Here's how the part is built. I have some questions about the finished solid (model axes, mm). Face numbers are marked on the shaded views. A direction names the side the tool comes from. Round coordinates to 2 decimals unless told otherwise and drop trailing zeros. Loops run counter-clockwise (first coordinate to the right, second up) from the corner with the lowest first, then second, coordinate; pieces in that order, holes last. Notation, with made-up numbers: (87.5, 84.25) - (116.5, 84.25) arc R13 cw to (116.5, 95.25) - close; hole circle Ø4 at (-17.75, -16.75). An arc over 180 degrees is marked (long way). Answer as a JSON object with one key per item and string values. Group by question number.
1) If we mould it in two halves opening along X, with no side actions, what happens to the marked faces 1, 2, 3 and 4? For each: pulls with the +X half, pulls with the -X half, needs draft (parallel to the pull), parting line crosses it, or undercut.
2) I want a section at C-C, the plane z = 27. Please give me the cut outline in (x, y), then the cut area to 3 significant figures.
3) I want a section at B-B, the plane z = 100. Please give me the cut outline in (x, y), then the cut area to 3 significant figures.
4) I want a section at A-A, the plane x = 18.5. Please give me the cut outline in (y, z).
5) Which directions (+Z, -Z, +X, -X, +Y, -Y) give clear straight access to the entire face, cutting with the end or side of a thin tool? Please do the marked faces 5, 6 and 7.
6) If I drill on line 1 along Z through (x, y) = (-45.5, -24.5); line 2 along Y through (x, z) = (-43.5, 98); line 3 along Y through (x, z) = (57, 90.5), over which ranges is the centre line in solid material (lowest first)? Write a range as [from, to].
7) Will these pins go through, and if not, where does the flat tip stop? P1, Ø1.5, axis at x = 18, z = 170, coming from the +Y side; P2, Ø12, axis at x = 94, y = -97, coming from the -Z side; P3, Ø3, axis at y = -313, z = 94, coming from the +X side; P4, Ø8, axis at x = 18.5, y = -164.5, coming from the +Z side.
8) I want a section at D-D, the plane x = 55. Please give me the cut outline in (y, z).
from build123d import *

# Parameters (mm, degrees)
SKETCH1_R           = 45
BOSS_EXTRUDE2_DEPTH = 200
SKETCH2_W           = 105
SKETCH2_H           = 318.049906591
CUT_EXTRUDE1_DEPTH  = 325.763563649
SKETCH3_R           = 50
BOSS_EXTRUDE3_DEPTH = 140
SKETCH4_R           = 50
BOSS_EXTRUDE4_DEPTH = 10
SKETCH5_R           = 40
BOSS_EXTRUDE5_DEPTH = 100


with BuildPart() as part:
    # Sketch1 → Boss-Extrude2 (new body)
    with BuildSketch(Plane.XY):
        with BuildLine():
            Line((140.402467833, -159.597532167), (-59.597532167, -159.597532167))
            Line((-59.597532167, -159.597532167), (-59.597532167, 40.402467833))
            ThreePointArc((-59.597532167, 40.402467833), (40.402467833, 140.402467833), (140.402467833, 40.402467833))
            Line((140.402467833, 40.402467833), (140.402467833, -159.597532167))
        make_face()
        with Locations((40.402467833, 40.402467833)):
            Circle(SKETCH1_R, mode=Mode.SUBTRACT)
    extrude(amount=BOSS_EXTRUDE2_DEPTH)

    # Sketch2 → Cut-Extrude1 (cut, through all)
    with BuildSketch(Plane(origin=(140.402467833, 0, 0), x_dir=(0, 0, -1), z_dir=(1, 0, 0))):
        with Locations((-100, 99.427421129)):
            Rectangle(SKETCH2_W, SKETCH2_H)
    extrude(amount=-CUT_EXTRUDE1_DEPTH, mode=Mode.SUBTRACT)

    # Sketch3 → Boss-Extrude3 (add)
    with BuildSketch(Plane.XZ.offset(159.597532167)):
        with Locations((40.402467833, 100)):
            Circle(SKETCH3_R)
    extrude(amount=BOSS_EXTRUDE3_DEPTH)

    # Sketch4 → Boss-Extrude4 (add)
    with BuildSketch(Plane.XZ.offset(299.597532167)):
        with Locations((40.402467833, 100)):
            Circle(SKETCH4_R)
    extrude(amount=BOSS_EXTRUDE4_DEPTH)

    # Sketch5 → Boss-Extrude5 (add)
    with BuildSketch(Plane.XZ.offset(309.597532167)):
        with Locations((40.402467833, 100)):
            Circle(SKETCH5_R)
    extrude(amount=BOSS_EXTRUDE5_DEPTH)


solid = part.part
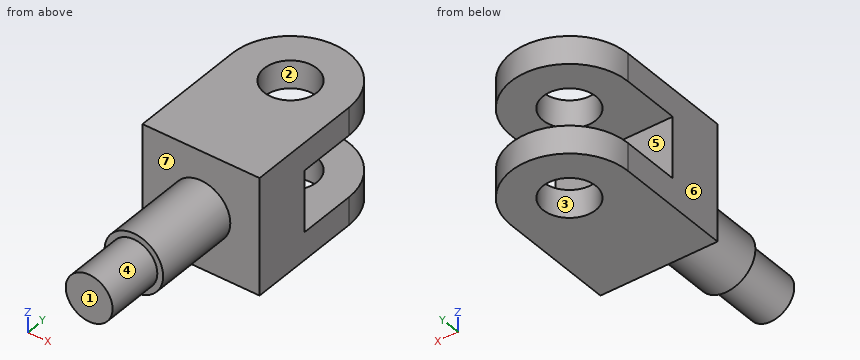
Outcome:
{
 "1": {"face 1": "needs draft", "face 2": "undercut", "face 3": "undercut", "face 4": "parting line crosses it"},
 "2": {"outline": "(-59.6, -159.6) - (140.4, -159.6) - (140.4, 40.4) arc R100 ccw to (-59.6, 40.4) - close; hole circle Ø90 at (40.4, 40.4)", "area": "49,300 mm^2"},
 "3": {"outline": "(-59.6, -159.6) - (-9.6, -159.6) - (-9.6, -309.6) - (0.4, -309.6) - (0.4, -409.6) - (80.4, -409.6) - (80.4, -309.6) - (90.4, -309.6) - (90.4, -159.6) - (140.4, -159.6) - (140.4, -59.6) - (-59.6, -59.6) - close", "area": "43,000 mm^2"},
 "4": {"outline": "(-409.6, 66.53) - (-309.6, 66.53) - (-309.6, 55.05) - (-159.6, 55.05) - (-159.6, 0) - (1.09, 0) - (1.09, 47.5) - (-59.6, 47.5) - (-59.6, 152.5) - (1.09, 152.5) - (1.09, 200) - (-159.6, 200) - (-159.6, 144.95) - (-309.6, 144.95) - (-309.6, 133.47) - (-409.6, 133.47) - close; (79.71, 0) - (137.97, 0) - (137.97, 47.5) - (79.71, 47.5) - close; (79.71, 152.5) - (137.97, 152.5) - (137.97, 200) - (79.71, 200) - close"},
 "5": {"face 5": "+X, -X, +Y", "face 6": "+Z, -Z, -X, +Y, -Y", "face 7": "-Y"},
 "6": {"line 1": "[0, 47.5], [152.5, 200]", "line 2": "[-159.6, -59.6]", "line 3": "[-409.6, -59.6]"},
 "7": {"P1": "y = 138.03", "P2": "z = 0", "P3": "x = 80.15", "P4": "z = 146.69"},
 "8": {"outline": "(-409.6, 62.76) - (-309.6, 62.76) - (-309.6, 52.18) - (-159.6, 52.18) - (-159.6, 0) - (-2.16, 0) - (-2.16, 47.5) - (-59.6, 47.5) - (-59.6, 152.5) - (-2.16, 152.5) - (-2.16, 200) - (-159.6, 200) - (-159.6, 147.82) - (-309.6, 147.82) - (-309.6, 137.24) - (-409.6, 137.24) - close; (82.97, 0) - (139.33, 0) - (139.33, 47.5) - (82.97, 47.5) - close; (82.97, 152.5) - (139.33, 152.5) - (139.33, 200) - (82.97, 200) - close"}
}
